Can you work these out from the drawing? Everything is in mm from the part's minimum corner. Coordinates: 2 decimals unless noted, no trailing zeros. Loops run counter-clockwise (first coordinate to the right, second up) from the corner with the lowest first, then second, coordinate; pieces in that order, holes last. Notation, with made-up numbers: (7, 13) - (64, 13) arc R19 ccw to (64, 24) - close; hole circle Ø11 at (-39.5, 78.25). An arc over 180 degrees is marked (long way). One line per question, with ' | ' between items. Start each with the question number.
1. I want a section at A-A, the plane y = 45. Write out the boundary of the cut face in (x, z).
2. We'd pull the mould along Z, two halves only. Please class the marked faces 1, 2 and 3: pulls with the +Z half, pulls with the -Z half, needs draft (parallel to the pull), parting line crosses it, or undercut.
3. I'm going to push flat-ended pins straight in: P1, Ø2, axis at x = 21, z = 23, coming from the -Y side; P2, Ø4, axis at y = 39.5, z = 28, coming from the +X side; P3, Ø10, axis at x = 19.5, z = 4.5, coming from the -Y side; P4, Ø5, axis at x = 55.5, y = 21, coming from the -Z side. Where does each tip first touch, or does it pass through?
4. I want a section at D-D, the plane z = 17. Write out the boundary of the cut face in (x, y).
5. I want a section at B-B, the plane x = 45. Write out the boundary of the cut face in (y, z).
6. I want a section at C-C, the plane z = 12. Write out the boundary of the cut face in (x, y), then the cut area to 3 significant figures.
7. Please list where these lines run through material, in increasing order: L1, parallel to Y at x = 45, z = 10; L2, parallel to Y at x = 59, z = 8.5; L3, parallel to X at y = 46, z = 10. Write a range as [from, to].
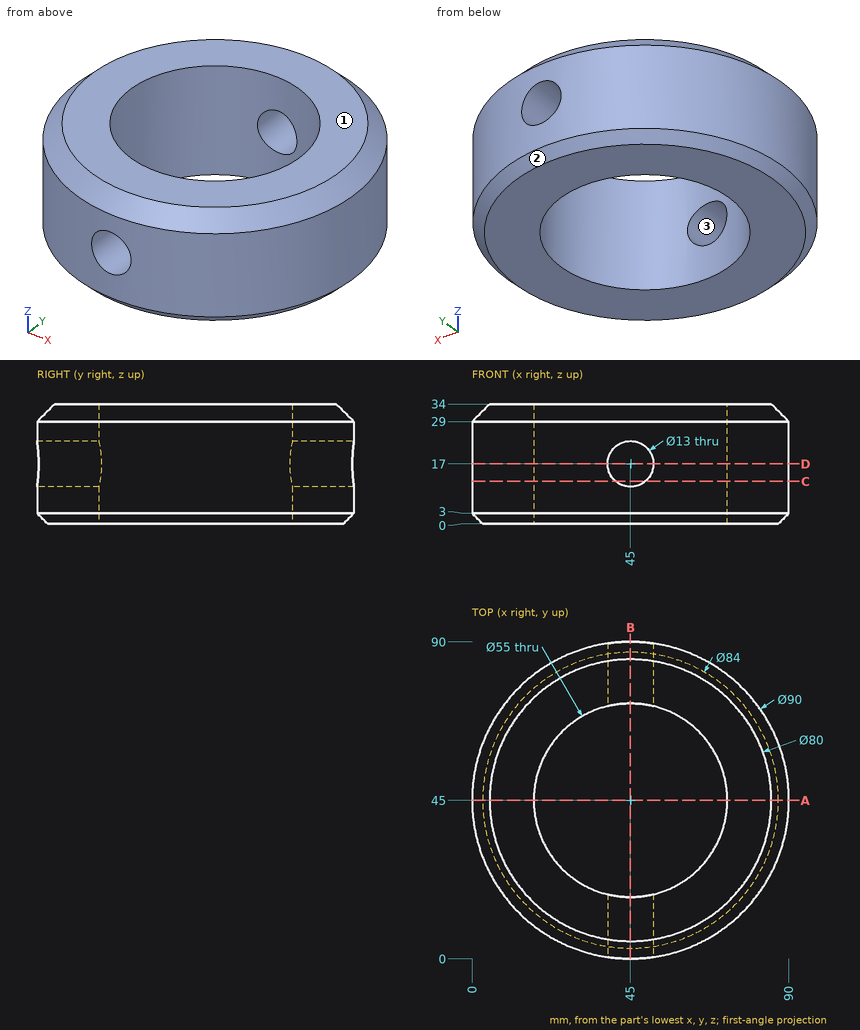
Results are:
1) outline: (0, 3) - (3, 0) - (17.5, 0) - (17.5, 34) - (5, 34) - (0, 29) - close; (72.5, 0) - (87, 0) - (90, 3) - (90, 29) - (85, 34) - (72.5, 34) - close
2) face 1: pulls with the +Z half | face 2: pulls with the -Z half | face 3: undercut
3) P1: stops at y = 6.32 | P2: stops at x = 89.86 | P3: stops at y = 4.94 | P4: stops at z = 0
4) outline: (38.5, 0.47) - (38.5, 18.28) arc R27.5 cw to (38.5, 71.72) - (38.5, 89.53) arc R45 ccw to start; (51.5, 0.47) arc R45 ccw to (51.5, 89.53) - (51.5, 71.72) arc R27.5 cw to (51.5, 18.28) - close
5) outline: (0, 3) - (3, 0) - (17.5, 0) - (17.5, 10.5) - (0, 10.5) - close; (0, 23.5) - (17.5, 23.5) - (17.5, 34) - (5, 34) - (0, 29) - close; (72.5, 0) - (87, 0) - (90, 3) - (90, 10.5) - (72.5, 10.5) - close; (72.5, 23.5) - (90, 23.5) - (90, 29) - (85, 34) - (72.5, 34) - close
6) outline: (40.85, 0.19) - (40.85, 17.82) arc R27.5 cw to (40.85, 72.18) - (40.85, 89.81) arc R45 ccw to start; (49.15, 0.19) arc R45 ccw to (49.15, 89.81) - (49.15, 72.18) arc R27.5 cw to (49.15, 17.82) - close | area: 3,690 mm2
7) L1: y = [0, 17.5], [72.5, 90] | L2: y = [2.23, 21.33], [68.67, 87.77] | L3: x = [0.01, 17.52], [72.48, 89.99]
